```python
from build123d import *

# Parameters (mm, degrees)
CHAMFER1_SIZE = 1


with BuildPart() as part:
    # Sketch1 → Revolve1 (revolve)
    with BuildSketch(Plane.XY, mode=Mode.PRIVATE) as revolve1_sk:
        Polygon((0, 0), (12.5, 0), (12.5, 35), (16, 35), (16, 365), (12.5, 365), (12.5, 400), (0, 400), align=None)
    revolve(revolve1_sk.sketch.rotate(Axis((0, 400, 0), (0, -1, 0)), 180), axis=Axis((0, 400, 0), (0, -1, 0)))

    # Chamfer1
    chamfer1_edges = [part.edges().sort_by_distance(p)[0] for p in [
        (12.5, 400, 0),
        (12.5, 0, 0),
    ]]
    chamfer(chamfer1_edges, length=CHAMFER1_SIZE)


solid = part.part
```
The listing builds one solid part. Answer for the finished solid, in the listing's coordinates (mm). A direction names the side the tool comes from. Give positions to 0.01 mm unless a question says otherwise; leave off trailing zeros. Write each loop counter-clockwise with the first axis right and the second up, starting at its lowest first coordinate (ties: lowest second). Pieces come first, ordered by that corner, then holes. Notation, with made-up numbers: (12.5, -28) - (23.5, -28) arc R20 cw to (23.5, -13) - close; hole circle Ø1 at (36.5, 28.5). An arc over 180 degrees is marked (long way). Use one line per item in the form item = value. Start each with the question number.
1) A tool of negligible diameter and unlimited length cuts with its end or side. For faces 1 (the face through (3.47, 202.31, 15.62)), 2 (the face through (-11.923, 18.238, -3.755)), 3 (the face through (10, 365, 8)), from which of +Z, -Z, +X, -X, +Y, -Y can it reach the whole face along a straight path? Write none if from no direction.
2) Consider line 1 along Y through (x, z) = (3, 14.5); line 2 along Z through (x, y) = (-1, 220); line 3 along Z through (x, y) = (8.5, 320). Determine where each line is inside the solid, lowest interval first. Write a range as from..to.
3) Find section B-B on z = 0. Determine the outline of the cut face in (x, y).
4) Flat-ended cylindrical pins translate along their axes: pin 1 Ø6 at (x, z) = (3.5, 4) entering from -Y; pin 2 Ø2 at (x, y) = (-12.5, 254) entering from +Z; pin 3 Ø6 at (x, y) = (-7.5, 289) entering from -Z; pin 4 Ø1.5 at (x, y) = (-4.5, 266.5) entering from -Z. Find the tip coordinate at first contact, or state that the pin passes through.
5) Find section C-C on y = 132. Determine the outline of the cut face in (x, z), plus the area to 3 significant figures.
6) Find section A-A on x = 0. Determine the outline of the cut face in (y, z), plus the area to 3 significant figures.
Geometry results:
q1.face_1 = +Y, -Y
q1.face_2 = -Y
q1.face_3 = +Y
q2.line_1 = 35..365
q2.line_2 = -15.97..15.97
q2.line_3 = -13.56..13.56
q3.outline = (-16, 35) - (-12.5, 35) - (-12.5, 1) - (-11.5, 0) - (11.5, 0) - (12.5, 1) - (12.5, 35) - (16, 35) - (16, 365) - (12.5, 365) - (12.5, 399) - (11.5, 400) - (-11.5, 400) - (-12.5, 399) - (-12.5, 365) - (-16, 365) - close
q4.pin_1 = 0
q4.pin_2 = 11.12
q4.pin_3 = -15.35
q4.pin_4 = -15.55
q5.outline = circle Ø32 at (0, 0)
q5.area = 804 mm2
q6.outline = (0, -11.5) - (1, -12.5) - (35, -12.5) - (35, -16) - (365, -16) - (365, -12.5) - (399, -12.5) - (400, -11.5) - (400, 11.5) - (399, 12.5) - (365, 12.5) - (365, 16) - (35, 16) - (35, 12.5) - (1, 12.5) - (0, 11.5) - close
q6.area = 12,300 mm2
